from build123d import *

# Parameters (mm, degrees)
SKETCH1_R           = 3
BOSS_EXTRUDE1_DEPTH = 20
SKETCH2_R           = 4.5
BOSS_EXTRUDE2_DEPTH = 3
CHAMFER1_SIZE       = 0.2


with BuildPart() as part:
    # Sketch1 → Boss-Extrude1 (new body)
    with BuildSketch(Plane.XY):
        Circle(SKETCH1_R)
    extrude(amount=BOSS_EXTRUDE1_DEPTH)

    # Sketch2 → Boss-Extrude2 (add)
    with BuildSketch(Plane.XY.offset(20)):
        Circle(SKETCH2_R)
    extrude(amount=BOSS_EXTRUDE2_DEPTH)

    # Chamfer1
    chamfer1_edges = [part.edges().sort_by_distance(p)[0] for p in [
        (-3, 0, 0),
        (-4.5, 0, 20),
        (-4.5, 0, 23),
    ]]
    chamfer(chamfer1_edges, length=CHAMFER1_SIZE)


solid = part.part
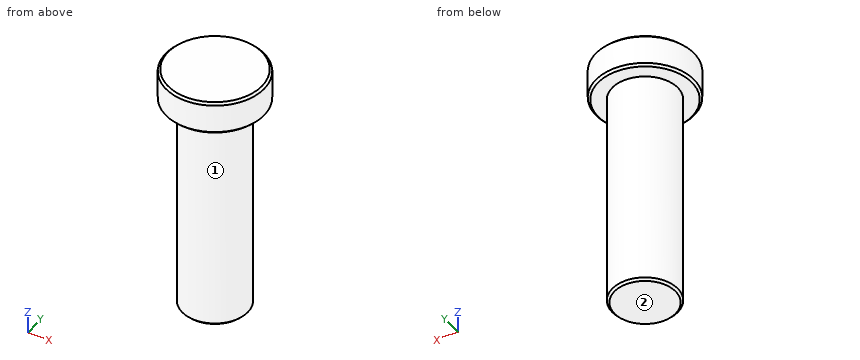
Geometry check sheet. Reference: the model listing, model coordinates, mm. Face numbers are marked on the shaded views. A direction names the side the tool comes from. Give positions to 0.01 mm unless a question says otherwise; leave off trailing zeros. Loops run counter-clockwise (first coordinate to the right, second up) from the corner with the lowest first, then second, coordinate; pieces in that order, holes last. Notation, with made-up numbers: (7, -8) -> (56, -8) arc R15 ccw to (56, 8) -> close; hole circle Ø5 at (26, -2.5). An arc over 180 degrees is marked (long way). Answer in a Markdown table with one row per item. Add a question column.
1) Gauge pin test, flat ends, axial feed: P1, Ø1.5, axis at y = -1.5, z = 13.5, coming from the -X side; P2, Ø4, axis at x = 0.5, z = 19, coming from the -Y side; P3, Ø5, axis at x = 3.5, z = 16.5, coming from the +Y side; P4, Ø3, axis at x = 3.5, z = 4.5, coming from the +Y side. Record the tip position at first contact, or that the pin passes through.
2) Cross-section at C-C on z = 6.75. Record the boundary of the cut face in (x, y).
3) Cross-section at A-A on x = 0. Record the boundary of the cut face in (y, z), and give its area (3 significant figures).
4) Material ranges on probe 1 along Z at (x, y) = (4, -0.5); probe 2 along Y at (x, z) = (0, 2.25); probe 3 along Y at (x, z) = (1.75, 14.25), recorded low to high. Write a range as from..to.
5) Set-up check for the marked faces 1 and 2: record each of +Z, -Z, +X, -X, +Y, -Y from which the full face is reachable in a straight line by a thin tool's end or side.
Outcome:
| question | item | result |
|---|---|---|
| 1 | P1 | stops at x = -2.9 |
| 1 | P2 | stops at y = -4.5 |
| 1 | P3 | stops at y = 2.83 |
| 1 | P4 | stops at y = 2.24 |
| 2 | outline | circle Ø6 at (0, 0) |
| 3 | outline | (-4.5, 20.2) -> (-4.3, 20) -> (-3, 20) -> (-3, 0.2) -> (-2.8, 0) -> (2.8, 0) -> (3, 0.2) -> (3, 20) -> (4.3, 20) -> (4.5, 20.2) -> (4.5, 22.8) -> (4.3, 23) -> (-4.3, 23) -> (-4.5, 22.8) -> close |
| 3 | area | 147 mm^2 |
| 4 | probe 1 | z = 20..23 |
| 4 | probe 2 | y = -3..3 |
| 4 | probe 3 | y = -2.44..2.44 |
| 5 | face 1 | -Z |
| 5 | face 2 | -Z, +X, -X, +Y, -Y |
